Geometry check sheet. Reference: the model listing, model coordinates, mm. Give positions to 0.01 mm unless a question says otherwise; leave off trailing zeros. Write each loop counter-clockwise with the first axis right and the second up, starting at its lowest first coordinate (ties: lowest second). Pieces come first, ordered by that corner, then holes. Notation, with made-up numbers: (58, -17.75) -> (105, -17.75) arc R12 ccw to (105, -10.75) -> close; hole circle Ø4 at (63, -7). An arc over 180 degrees is marked (long way). Write item = value, one per line. Start each with the question number.
1. Thickness scan on line 1 along Y through (x, z) = (147.5, 1.65); line 2 along Y through (x, z) = (-94, 1); line 3 along Y through (x, z) = (20.5, 1.8). Record the ranges inside material, lowest first.
2. Cross-section at A-A, the plane y = 26.5. Record the cut outline in (x, z), plus the area to 3 significant figures.
3. Cross-section at B-B, the plane x = 15.5. Record the cut outline in (y, z), plus the area to 3 significant figures.
4. Cross-section at C-C, the plane x = 144. Record the cut outline in (y, z) (3 decimals), plus the area to 3 significant figures.
5. Cross-section at D-D, the plane x = -181.5. Record the cut outline in (y, z), plus the area to 3 significant figures.
6. Depth check by flat-ended pin: P1, Ø3, axis at x = -135.5, z = 2, coming from the +Y side; P2, Ø2, axis at x = 61.5, z = 0.5, coming from the -Y side; P3, Ø1, axis at y = -5.5, z = 4, coming from the -X side. Enter the tip coordinate at first touch or a pass-through.
```python
from build123d import *

# Parameters (mm, degrees)
EXTRUDE_1_DEPTH     = 5
CUT_EXTRUDE_1_DEPTH = 606
SKETCH_4_W          = 70
SKETCH_4_H          = 5.4
SKETCH_4_W_2        = 5.4
SKETCH_4_H_2        = 70
CUT_EXTRUDE_2_DEPTH = 10


with BuildPart() as part:
    # 草图1 → 凸台-拉伸1 (new body)
    with BuildSketch(Plane.XY):
        Polygon((159.099025767, 159.099025767), (0, 225), (-159.099025767, 159.099025767), (-225, 0), (-159.099025767, -159.099025767), (0, -225), (159.099025767, -159.099025767), (225, 0), align=None)
    extrude(amount=EXTRUDE_1_DEPTH)

    # 草图2 → 切除-拉伸1 (cut)
    with BuildSketch(Plane.XY.offset(5)):
        Polygon((0, 170.880389985), (-120.83068253, 120.83068253), (-170.880389985, 0), (-120.83068253, -120.83068253), (0, -170.880389985), (120.83068253, -120.83068253), (170.880389985, 0), (120.83068253, 120.83068253), align=None)
    extrude(amount=-CUT_EXTRUDE_1_DEPTH, mode=Mode.SUBTRACT)

    # 草图4 → 切除-拉伸2 (cut)
    with BuildSketch(Plane.XY.offset(5)):
        Polygon((185.756951418, -181.938574799), (136.259476735, -132.441100116), (132.441100116, -136.259476735), (181.938574799, -185.756951418), align=None)
        with Locations((225, 0)):
            Rectangle(SKETCH_4_W, SKETCH_4_H)
        with Locations((0, -225)):
            Rectangle(SKETCH_4_W_2, SKETCH_4_H_2)
        Polygon((-181.938574799, -185.756951418), (-132.441100116, -136.259476735), (-136.259476735, -132.441100116), (-185.756951418, -181.938574799), align=None)
        with Locations((-225, 0)):
            Rectangle(SKETCH_4_W, SKETCH_4_H)
        Polygon((-185.756951418, 181.938574799), (-136.259476735, 132.441100116), (-132.441100116, 136.259476735), (-181.938574799, 185.756951418), align=None)
        with Locations((0, 225)):
            Rectangle(SKETCH_4_W_2, SKETCH_4_H_2)
        Polygon((181.938574799, 185.756951418), (132.441100116, 136.259476735), (136.259476735, 132.441100116), (185.756951418, 181.938574799), align=None)
    extrude(amount=-CUT_EXTRUDE_2_DEPTH, mode=Mode.SUBTRACT)


solid = part.part
```
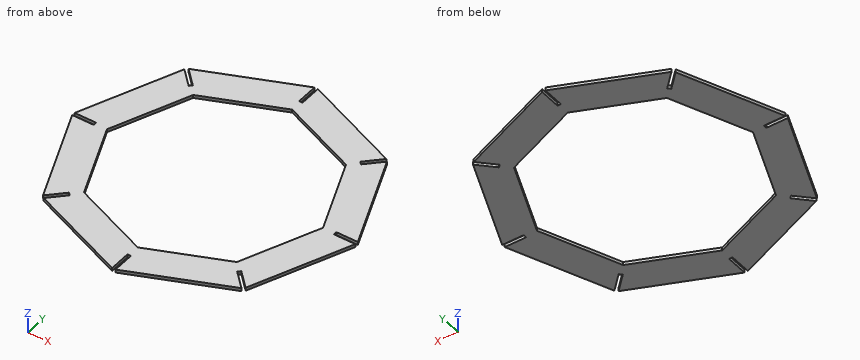
Answers:
q1.line_1 = -163.9 to -151.32, -143.68 to -56.45, 56.45 to 143.68, 151.32 to 163.9
q1.line_2 = -186.06 to -131.94, 131.94 to 186.06
q1.line_3 = -216.51 to -162.39, 162.39 to 216.51
q2.outline = (-214.02, 0) -> (-159.9, 0) -> (-159.9, 5) -> (-214.02, 5) -> close; (159.9, 0) -> (214.02, 0) -> (214.02, 5) -> (159.9, 5) -> close
q2.area = 541 mm^2
q3.outline = (-218.58, 0) -> (-164.46, 0) -> (-164.46, 5) -> (-218.58, 5) -> close; (164.46, 0) -> (218.58, 0) -> (218.58, 5) -> (164.46, 5) -> close
q3.area = 541 mm^2
q4.outline = (-165.353, 0) -> (-147.818, 0) -> (-147.818, 5) -> (-165.353, 5) -> close; (-140.182, 0) -> (-64.895, 0) -> (-64.895, 5) -> (-140.182, 5) -> close; (64.895, 0) -> (140.182, 0) -> (140.182, 5) -> (64.895, 5) -> close; (147.818, 0) -> (165.353, 0) -> (165.353, 5) -> (147.818, 5) -> close
q4.area = 928 mm^2
q5.outline = (-105.02, 0) -> (105.02, 0) -> (105.02, 5) -> (-105.02, 5) -> close
q5.area = 1,050 mm^2
q6.P1 = 169.5
q6.P2 = -199.94
q6.P3 = -222.93
